Part model, mm, in its own coordinate system. Round coordinates to 2 decimals unless told otherwise and drop trailing zeros. Order: outer loops, then holes, each group sorted by start corner. A loop starts at its lowest first (then second) coordinate and runs counter-clockwise, first axis right, second up. Notation, with made-up numbers: (81, 26.5) -> (88, 26.5) arc R30 cw to (88, 58.5) -> close; hole circle Ø3 at (21, 66). An arc over 180 degrees is marked (long way). Use CSV: the item, a comma, the result in double quotes.
```python
from build123d import *

# Parameters (mm, degrees)
BASE_EXTRUDE_DEPTH = 9
FILLET1_R          = 0.6


with BuildPart() as part:
    # Sketch1 → Base-Extrude (new body)
    with BuildSketch(Plane.XY):
        with BuildLine():
            Line((-73, 7), (73, 7))
            ThreePointArc((73, 7), (80, 0), (73, -7))
            Line((73, -7), (-73, -7))
            ThreePointArc((-73, -7), (-80, 0), (-73, 7))
        make_face()
    extrude(amount=BASE_EXTRUDE_DEPTH)

    # Fillet1
    fillet1_edges = [part.edges().sort_by_distance(p)[0] for p in [
        (80, 0, 9),
        (0, 7, 9),
        (-80, 0, 9),
        (0, 7, 0),
        (80, 0, 0),
        (0, -7, 0),
        (-80, 0, 0),
        (0, -7, 9),
    ]]
    fillet(fillet1_edges, radius=FILLET1_R)


solid = part.part
```
(1) Cut at A-A, the plane z = 4.5. Give the cut face in (x, y), then the cut area to 3 significant figures.
Reply:
outline,"(-73, -7) -> (73, -7) arc R7 ccw to (73, 7) -> (-73, 7) arc R7 ccw to start"
area,"2,200 mm2"
(2) Drop flat-ended pins along their axis: P1, Ø1.5, axis at y = 1.5, z = 2.5, coming from the -X side; P2, Ø1, axis at y = 3, z = 1.5, coming from the +X side. Give the stop position or say it passes through.
Reply:
P1,"x = -79.96"
P2,"x = 79.54"
(3) Probe probe 1 along X at (y, z) = (-0.25, 7.25); probe 2 along X at (y, z) = (-4, 6.75). List the from-to ranges inside material, lowest first. Write a range as [from, to].
Reply:
probe 1,"[-80, 80]"
probe 2,"[-78.74, 78.74]"
